Can you work these out from the model? Positions are in its coordinate system, mm. A direction names the side the tool comes from. Give positions to 0.01 mm unless a question says otherwise; leave off trailing zeros. Order: outer loops, then holes, each group sorted by start corner. A loop starts at its lowest first (then second) coordinate and runs counter-clockwise, first axis right, second up. Notation, with made-up numbers: M 26.25,23 L 73.25,23 A35 cw 73.25,58 Z; hole C 60.5,44.5 d1. An arc over 180 degrees is marked long. Answer as a JSON object with one key per item and string values.
```python
from build123d import *

# Parameters (mm, degrees)
SKETCH_1_W               = 81
SKETCH_1_H               = 125
EXTRUDE_1_DEPTH          = 14
CUT_EXTRUDE_1_DEPTH      = 150.606149606
CUT_EXTRUDE_2_REACH      = 145.948
CUT_EXTRUDE_2_END_RADIUS = 7
SKETCH_4_R               = 3.25
HOLE_WIZARD_M8_1_D       = 6.8
HOLE_WIZARD_M8_1_DEPTH   = 22.25
HOLE_WIZARD_M8_1_TIP     = 2.042926105
SKETCH_11_R              = 2.75
CUT_EXTRUDE_3_DEPTH      = 150.606149699


with BuildPart() as part:
    # 草图1 → 凸台-拉伸1 (new body)
    with BuildSketch(Plane.XY):
        with Locations((40.5, -62.5)):
            Rectangle(SKETCH_1_W, SKETCH_1_H)
    extrude(amount=EXTRUDE_1_DEPTH)

    # 草图2 → 切除-拉伸1 (cut, through all)
    with BuildSketch(Plane.XY.offset(14)):
        with BuildLine():
            Line((33.5, -70), (33.5, -40))
            ThreePointArc((33.5, -40), (40.5, -33), (47.5, -40))
            Line((47.5, -40), (47.5, -70))
            ThreePointArc((47.5, -70), (40.5, -77), (33.5, -70))
        make_face()
    extrude(amount=-CUT_EXTRUDE_1_DEPTH, mode=Mode.SUBTRACT)

    # 切除-拉伸2: up to this cylinder (the profile starts outside it)
    cut_extrude_2_end = Plane(origin=(40.5, -70, 7), z_dir=(0, 0, 1)) * Cylinder(CUT_EXTRUDE_2_END_RADIUS, 306.896, mode=Mode.PRIVATE)
    # 草图4 → 切除-拉伸2 (cut, up to the surface)
    with BuildSketch(Plane(origin=(70, -125, 0), x_dir=(0, 0, -1), z_dir=(0, -1, 0)), mode=Mode.PRIVATE) as cut_extrude_2_sk1:
        with Locations((-7, -29)):
            Circle(SKETCH_4_R)
    cut_extrude_2_tool1 = extrude(cut_extrude_2_sk1.sketch, amount=-CUT_EXTRUDE_2_REACH, mode=Mode.PRIVATE) - cut_extrude_2_end
    add(cut_extrude_2_tool1.solids().sort_by_distance((41, -125, 7))[0], mode=Mode.SUBTRACT)

    # M8 螺纹孔1
    with Locations(Plane(origin=(0, 0, 0), x_dir=(1, 0, 0), z_dir=(0, 1, 0))):
        with Locations((68, -7), (13, -7)):
            Hole(HOLE_WIZARD_M8_1_D / 2, depth=HOLE_WIZARD_M8_1_DEPTH)
            with Locations((0, 0, -(HOLE_WIZARD_M8_1_DEPTH + HOLE_WIZARD_M8_1_TIP / 2))):  # 118° drill point
                Cone(0, HOLE_WIZARD_M8_1_D / 2, HOLE_WIZARD_M8_1_TIP, mode=Mode.SUBTRACT)

    # 草图11 → 切除-拉伸3 (cut, through all)
    with BuildSketch(Plane.XY.offset(14)):
        with Locations((15.5, -120)):
            Circle(SKETCH_11_R)
        with Locations((65.5, -120)):
            Circle(SKETCH_11_R)
    extrude(amount=-CUT_EXTRUDE_3_DEPTH, mode=Mode.SUBTRACT)


solid = part.part
```
1) For faces 1 (the face through (40.35, -33, 7.1)), 2 (the face through (31, -62, 0)), 3 (the face through (37.827, -100.799, 7.705)), 4 (the face through (64.86, -11.28, 8.3)), which set-ups out of +Z, -Z, +X, -X, +Y, -Y let a thin tool reach every point of the face, with its end or its side?
Results found:
{"face 1": "+Z, -Z", "face 2": "-Z, +X, -X, +Y, -Y", "face 3": "-Y", "face 4": "+Y"}
2) I want a section at A-A on y = -120. Write out the boundary of the cut face in (x, z), and give its area (3 significant figures).
Results found:
{"outline": "M 0,0 L 12.75,0 L 12.75,14 L 0,14 Z; M 18.25,0 L 62.75,0 L 62.75,14 L 18.25,14 Z; M 68.25,0 L 81,0 L 81,14 L 68.25,14 Z; hole C 41,7 d6.5", "area": "947 mm²"}
3) Thinking about a two-plate mould opening in X: for faces 5 (the face through (13.74, -11.28, 10.32)), 6 (the face through (81, -63, 7)), 7 (the face through (40, 0, 7)), which applies, pulls with the +X half, pulls with the -X half, needs draft (parallel to the pull), parting line crosses it, or undercut?
Results found:
{"face 5": "undercut", "face 6": "pulls with the +X half", "face 7": "needs draft"}
4) I want a section at C-C on y = -9. Write out the boundary of the cut face in (x, z).
Results found:
{"outline": "M 0,0 L 81,0 L 81,14 L 0,14 Z; hole C 13,7 d6.8; hole C 68,7 d6.8"}
5) I need wall thicknesses on L1, parallel to X at y = -104, z = 7; L2, parallel to Z at x = 68, y = -5.5; L3, parallel to X at y = -56.5, z = 12.25. Which ranges of each line are inside material? Lowest first, please.
Results found:
{"L1": "x = 0 to 37.75, 44.25 to 81", "L2": "z = 0 to 3.6, 10.4 to 14", "L3": "x = 0 to 33.5, 47.5 to 81"}
6) I want a section at D-D on y = -95.5. Write out the boundary of the cut face in (x, z), and give its area (3 significant figures).
Results found:
{"outline": "M 0,0 L 81,0 L 81,14 L 0,14 Z; hole C 41,7 d6.5", "area": "1,100 mm²"}
7) I want a section at B-B on x = 39. Write out the boundary of the cut face in (y, z).
Results found:
{"outline": "M -125,0 L -76.84,0 L -76.84,4.44 L -125,4.44 Z; M -125,9.56 L -76.84,9.56 L -76.84,14 L -125,14 Z; M -33.16,0 L 0,0 L 0,14 L -33.16,14 Z"}
8) I'm going to push a flat-ended pin straight in: pin 1 Ø5 at (x, y) = (65.5, -120) entering from -Z. Where does the tip first touch, or does it pass through?
Results found:
{"pin 1": "passes through"}
